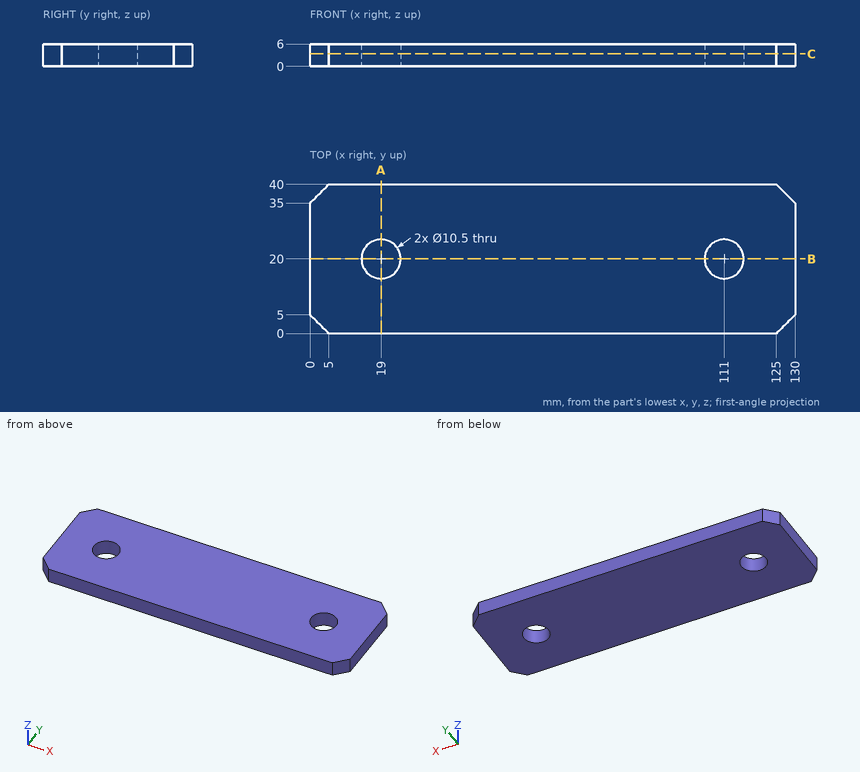
Here's the drawing with two shaded views (mm, measured from the low corner). I have some questions. Round coordinates to 2 decimals unless told otherwise and drop trailing zeros. Write each loop counter-clockwise with the first axis right and the second up, starting at its lowest first coordinate (ties: lowest second). Pieces come first, ordered by that corner, then holes. Notation, with made-up numbers: M 65,42 L 92,42 A35 cw 92,75 Z; hole C -14.75,-18 d10. An arc over 180 degrees is marked long. Use CSV: the item, a comma, the result in double quotes.
(1) I need wall thicknesses on line 1 along Y through (x, z) = (111, 2.5); line 2 along Y through (x, z) = (22, 1.1). Which ranges of each line are inside material? Lowest first, please.
Check values:
line 1,"0 to 14.75, 25.25 to 40"
line 2,"0 to 15.69, 24.31 to 40"
(2) Imagine slicing it at C-C (z = 3.35). Write out the boundary of the cut face in (x, y).
Check values:
outline,"M 0,5 L 5,0 L 125,0 L 130,5 L 130,35 L 125,40 L 5,40 L 0,35 Z; hole C 19,20 d10.5; hole C 111,20 d10.5"
(3) Imagine slicing it at B-B (y = 20). Write out the boundary of the cut face in (x, z).
Check values:
outline,"M 0,0 L 13.75,0 L 13.75,6 L 0,6 Z; M 24.25,0 L 105.75,0 L 105.75,6 L 24.25,6 Z; M 116.25,0 L 130,0 L 130,6 L 116.25,6 Z"
(4) Imagine slicing it at A-A (x = 19). Write out the boundary of the cut face in (y, z).
Check values:
outline,"M 0,0 L 14.75,0 L 14.75,6 L 0,6 Z; M 25.25,0 L 40,0 L 40,6 L 25.25,6 Z"
(5) I'm going to push a flat-ended pin straight in: pin 1 (6.5 mm diameter, centred on x = 111, y = 20, fed in from -Z). Where does the tip first touch, or does it pass through?
Check values:
pin 1,"through"
